Here's the drawing with two shaded views (mm, measured from the low corner). I have some questions. Coordinates: 2 decimals unless noted, no trailing zeros. Loops run counter-clockwise (first coordinate to the right, second up) from the corner with the lowest first, then second, coordinate; pieces in that order, holes last. Notation, with made-up numbers: (20, 45.5) - (65, 45.5) arc R26 cw to (65, 74.5) - close; hole circle Ø11 at (83.5, -3). An arc over 180 degrees is marked (long way). One line per item, written item: value. Start each with the question number.
(1) I'm going to push a flat-ended pin straight in: P1, Ø3, axis at x = 214.5, z = 11, coming from the -Y side. Where does the tip first touch, or does it pass through?
(2) If we section it at A-A on y = 55: Write out the boundary of the cut face in (x, z), then the cut area to 3 significant figures.
(3) If we section it at C-C on x = 296: Write out the boundary of the cut face in (y, z), then the cut area to 3 significant figures.
(4) If we section it at B-B on y = 87: Write out the boundary of the cut face in (x, z), then the cut area to 3 significant figures.
(5) If we section it at D-D on y = 223: Write out the boundary of the cut face in (x, z).
(6) If I drill on line 1 along Y through (x, z) = (60, 7.5); line 2 along X through (y, z) = (215.5, 6.25); line 3 along X through (y, z) = (78, 1), over which ranges is the centre line in solid material (lowest first)? Write a range as from..to.
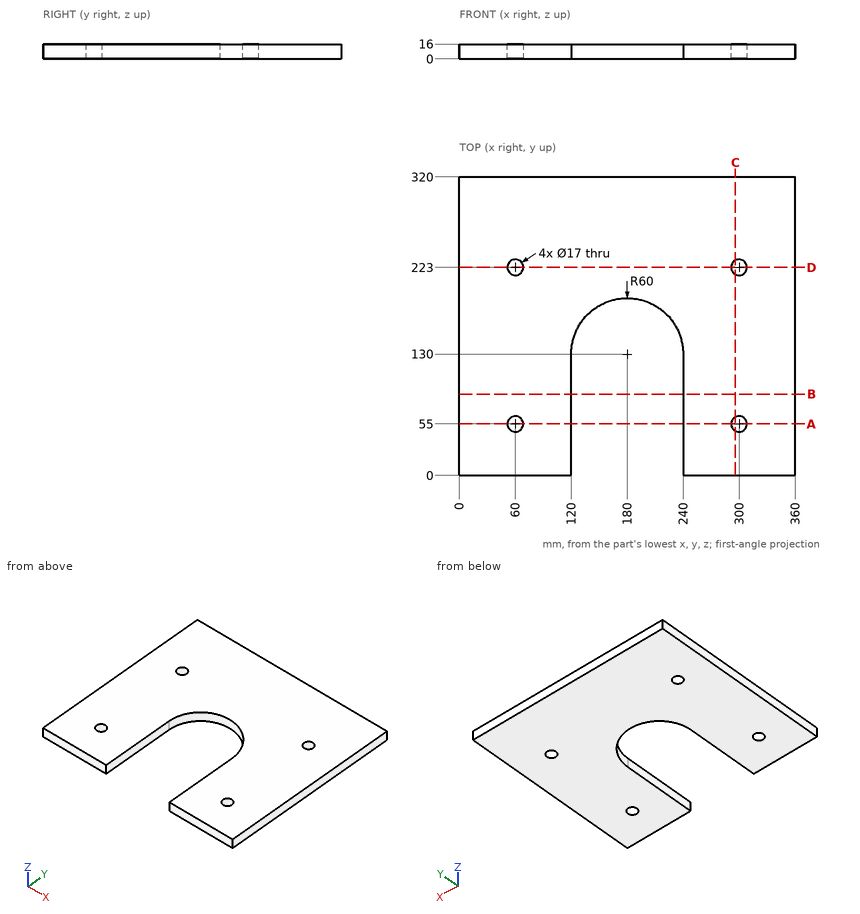
Values:
1. P1: stops at y = 178
2. outline: (0, 0) - (51.5, 0) - (51.5, 16) - (0, 16) - close; (68.5, 0) - (120, 0) - (120, 16) - (68.5, 16) - close; (240, 0) - (291.5, 0) - (291.5, 16) - (240, 16) - close; (308.5, 0) - (360, 0) - (360, 16) - (308.5, 16) - close
2. area: 3,300 mm2
3. outline: (0, 0) - (47.5, 0) - (47.5, 16) - (0, 16) - close; (62.5, 0) - (215.5, 0) - (215.5, 16) - (62.5, 16) - close; (230.5, 0) - (320, 0) - (320, 16) - (230.5, 16) - close
3. area: 4,640 mm2
4. outline: (0, 0) - (120, 0) - (120, 16) - (0, 16) - close; (240, 0) - (360, 0) - (360, 16) - (240, 16) - close
4. area: 3,840 mm2
5. outline: (0, 0) - (51.5, 0) - (51.5, 16) - (0, 16) - close; (68.5, 0) - (291.5, 0) - (291.5, 16) - (68.5, 16) - close; (308.5, 0) - (360, 0) - (360, 16) - (308.5, 16) - close
6. line 1: y = 0..46.5, 63.5..214.5, 231.5..320
6. line 2: x = 0..56, 64..296, 304..360
6. line 3: x = 0..120, 240..360
